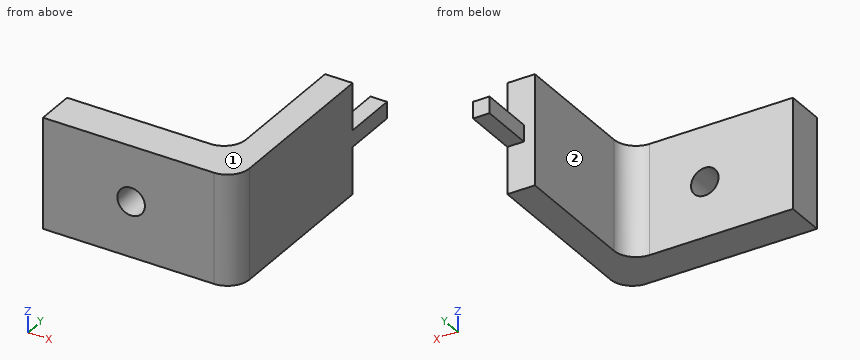
from build123d import *

# Parameters (mm, degrees)
BOSS_EXTRUDE1_DEPTH   = 10
SKETCH2_W             = 1.5
SKETCH2_H             = 5
BOSS_EXTRUDE2_DEPTH   = 1.5
FILLET1_R             = 2
M3_TAPPED_HOLE1_D     = 2.5
M3_TAPPED_HOLE1_DEPTH = 8.5
M3_TAPPED_HOLE1_TIP   = 0.751075774


with BuildPart() as part:
    # Sketch1 → Boss-Extrude1 (new body)
    with BuildSketch(Plane.XY):
        Polygon((0, 0), (17.5, 0), (17.5, 17), (15, 17), (15, 3.5), (0, 3.5), align=None)
    extrude(amount=BOSS_EXTRUDE1_DEPTH)

    # Sketch2 → Boss-Extrude2 (add)
    with BuildSketch(Plane(origin=(17.5, 0, 0), x_dir=(0, 0, -1), z_dir=(1, 0, 0))):
        with Locations((-5, 19.5)):
            Rectangle(SKETCH2_W, SKETCH2_H)
    extrude(amount=-BOSS_EXTRUDE2_DEPTH)

    # Fillet1
    fillet1_edges = [part.edges().sort_by_distance(p)[0] for p in [
        (15, 3.5, 5),
        (17.5, 0, 5),
    ]]
    fillet(fillet1_edges, radius=FILLET1_R)

    # M3 Tapped Hole1
    with Locations(Plane(origin=(0, 3.5, 0), x_dir=(1, 0, 0), z_dir=(0, 1, 0))):
        with Locations((8, -5)):
            Hole(M3_TAPPED_HOLE1_D / 2, depth=M3_TAPPED_HOLE1_DEPTH)
            with Locations((0, 0, -(M3_TAPPED_HOLE1_DEPTH + M3_TAPPED_HOLE1_TIP / 2))):  # 118° drill point
                Cone(0, M3_TAPPED_HOLE1_D / 2, M3_TAPPED_HOLE1_TIP, mode=Mode.SUBTRACT)


solid = part.part
For this review, take the finished solid that the model builds, in its own axes (mm). Face numbers are marked on the shaded views. A direction names the side the tool comes from. Give positions to 0.01 mm unless a question says otherwise; leave off trailing zeros. Loops run counter-clockwise (first coordinate to the right, second up) from the corner with the lowest first, then second, coordinate; pieces in that order, holes last.
Item 1: For line 1 along Z through (x, y) = (8, 2.65); line 2 along X through (y, z) = (2.4, 5); line 3 along X through (y, z) = (15.75, 8.75), list the stretches that pass through material, from the lowest coordinate up.
Item 2: Take a section at B-B, the plane z = 5. State the section outline as (x, y) points, and give its area (4 significant figures).
Item 3: Insertion check: pin 1 (3 mm diameter, centred on y = 12, z = 5, fed in from -X); pin 2 (1.6 mm diameter, centred on x = 16.5, y = 20, fed in from -Z); pin 3 (3 mm diameter, centred on x = 7.5, z = 3, fed in from +Y). Each pin has a flat end and moves straight along its axis. Give the tip position at first contact, or say it passes through.
Item 4: Take a section at A-A, the plane x = 8. State the section outline as (y, z) points, and give its area (4 significant figures).
Item 5: Take a section at D-D, the plane y = 19.75. State the section outline as (x, z) points.
Item 6: Take a section at C-C, the plane z = 7.5. State the section outline as (x, y) points, and give its area (3 significant figures).
Item 7: Tool access review of the marked faces 1 and 2: name each direction out of +Z, -Z, +X, -X, +Y, -Y from which nothing blocks a thin tool from reaching the whole face with its end or side.
Calculated:
1. line 1: z = 0 to 3.75, 6.25 to 10
1. line 2: x = 0 to 6.75, 9.25 to 17.5
1. line 3: x = 15 to 17.5
2. outline: (0, 0) - (6.75, 0) - (6.75, 3.5) - (0, 3.5) - close; (9.25, 0) - (15.5, 0) arc R2 ccw to (17.5, 2) - (17.5, 22) - (16, 22) - (16, 17) - (15, 17) - (15, 5.5) arc R2 cw to (13, 3.5) - (9.25, 3.5) - close
2. area: 93.75 mm2
3. pin 1: stops at x = 15
3. pin 2: stops at z = 4.25
3. pin 3: stops at y = 3.5
4. outline: (0, 0) - (3.5, 0) - (3.5, 3.75) - (0, 3.75) - close; (0, 6.25) - (3.5, 6.25) - (3.5, 10) - (0, 10) - close
4. area: 26.25 mm2
5. outline: (16, 4.25) - (17.5, 4.25) - (17.5, 5.75) - (16, 5.75) - close
6. outline: (0, 0) - (15.5, 0) arc R2 ccw to (17.5, 2) - (17.5, 17) - (15, 17) - (15, 5.5) arc R2 cw to (13, 3.5) - (0, 3.5) - close
6. area: 95.0 mm2
7. face 1: +Z, +X, -X, +Y, -Y
7. face 2: +Z, -Z, -X, +Y
